from build123d import *

# Parameters (mm, degrees)
BASE_BODY_EXTRUDE_DEPTH         = 25
FLANGE_END_ROUNDS_R12_5_R       = 12.5
EDGE_FILLETS_R6_R               = 6
FLANGE_BOLT_HOLES_2X_DEPTH      = 64.442887702
FLANGE_BOLT_HOLES_2X_DEPTH_BACK = 64.442887702
FLANGE_HOLES_SKETCH_R           = 5
FORK_SLOT_REACH                 = 112.567
FORK_SLOT_DIRECTION_2_DEPTH     = 111.566721937


with BuildPart() as part:
    # Base Profile Sketch → Base Body Extrude (new, symmetric)
    with BuildSketch(Plane.XY):
        with BuildLine():
            Line((50, 40), (50, 0))
            Line((50, 0), (20, 0))
            ThreePointArc((20, 0), (0, 20), (-20, 0))
            Line((-20, 0), (-50, 0))
            Line((-50, 0), (-50, 10))
            Line((-50, 10), (-28.284271247, 10))
            ThreePointArc((-28.284271247, 10), (0, 30), (28.284271247, 10))
            Line((28.284271247, 10), (40, 10))
            Line((40, 10), (40, 40))
            Line((40, 40), (50, 40))
        make_face()
    extrude(amount=BASE_BODY_EXTRUDE_DEPTH, both=True)

    # Flange End Rounds R12.5
    flange_end_rounds_r12_5_edges = [part.edges().sort_by_distance(p)[0] for p in [
        (-50, 5, 25),
        (-50, 5, -25),
    ]]
    fillet(flange_end_rounds_r12_5_edges, radius=FLANGE_END_ROUNDS_R12_5_R)

    # Edge Fillets R6
    edge_fillets_r6_edges = [part.edges().sort_by_distance(p)[0] for p in [
        (45, 40, -25),
        (45, 40, 25),
    ]]
    fillet(edge_fillets_r6_edges, radius=EDGE_FILLETS_R6_R)

    # Flange Holes Sketch → Flange Bolt Holes 2x (cut, two sides: drawn at the far end of the back side and taken through both)
    with BuildSketch(Plane(origin=(0, 10, 0), x_dir=(1, 0, 0), z_dir=(0, 1, 0)).offset(-FLANGE_BOLT_HOLES_2X_DEPTH_BACK)):
        with Locations(Location((-37.5, -12.5, 0), (0, 0, 180))):
            Circle(FLANGE_HOLES_SKETCH_R)
        with Locations(Location((-37.5, 12.5, 0), (0, 0, 180))):
            Circle(FLANGE_HOLES_SKETCH_R)
    extrude(amount=FLANGE_BOLT_HOLES_2X_DEPTH + FLANGE_BOLT_HOLES_2X_DEPTH_BACK, mode=Mode.SUBTRACT)

    # Fork Slot Sketch → Fork Slot (cut, up to next)
    with BuildSketch(Plane(origin=(50, 0, 0), x_dir=(0, 0, -1), z_dir=(1, 0, 0)), mode=Mode.PRIVATE) as fork_slot_sk1:
        with BuildLine():
            Line((7.5, 40), (7.5, 25))
            ThreePointArc((7.5, 25), (0, 17.5), (-7.5, 25))
            Line((-7.5, 25), (-7.5, 40))
            Line((-7.5, 40), (7.5, 40))
        make_face()
    fork_slot_tool1 = extrude(fork_slot_sk1.sketch, amount=-FORK_SLOT_REACH, mode=Mode.PRIVATE) & part.part
    add(fork_slot_tool1.solids().sort_by_distance((50, 29.487689, 0))[0], mode=Mode.SUBTRACT)

    # Fork Slot Sketch → Fork Slot direction 2 (cut)
    with BuildSketch(Plane(origin=(50, 0, 0), x_dir=(0, 0, -1), z_dir=(1, 0, 0))):
        with BuildLine():
            Line((7.5, 40), (7.5, 25))
            ThreePointArc((7.5, 25), (0, 17.5), (-7.5, 25))
            Line((-7.5, 25), (-7.5, 40))
            Line((-7.5, 40), (7.5, 40))
        make_face()
    extrude(amount=FORK_SLOT_DIRECTION_2_DEPTH, mode=Mode.SUBTRACT)


solid = part.part
Read the model definition and answer for the solid it produces. Units are mm, in the model's axes. A direction names the side the tool comes from. Give positions to 0.01 mm unless a question says otherwise; leave off trailing zeros. Write each loop counter-clockwise with the first axis right and the second up, starting at its lowest first coordinate (ties: lowest second). Pieces come first, ordered by that corner, then holes. Notation, with made-up numbers: (75.5, 11) - (91.5, 11) arc R19 ccw to (91.5, 20) - close; hole circle Ø1 at (67, 19.25). An arc over 180 degrees is marked (long way). Answer in a Markdown table with one row per item. Add a question column.
Item 1: Determine the mould class of faces 1 (the face through (45.07, 38.196, 23.289)), 2 (the face through (0, 20, 0)), 3 (the face through (-32.505, 4.93, 12.72)) for opening direction Z: pulls with the +Z half, pulls with the -Z half, needs draft (parallel to the pull), parting line crosses it, or undercut.
Item 2: Section A-A, the plane z = 8.5 is taken. Write down the section's boundary in (x, y), and give its area (3 significant figures).
Item 3: Section B-B, the plane y = 31 is taken. Write down the section's boundary in (x, z), and give its area (3 significant figures).
Item 4: A tool of negligible diameter and unlimited length cuts with its end or side. For faces 4 (the face through (45.07, 38.289, -23.196)), 5 (the face through (45, 33, -7.5)), 6 (the face through (40, 18, 6)), from which of +Z, -Z, +X, -X, +Y, -Y can it reach the whole face along a straight path? Write none if from no direction.
Item 5: Section C-C, the plane x = -36 is taken. Write down the section's boundary in (y, z), and give its area (3 significant figures).
Item 6: Section D-D, the plane y = 22.5 is taken. Write down the section's boundary in (x, z).
Item 7: Find the intervals of material crossed by L1, parallel to Z at x = -37.5, y = 6.5; L2, parallel to X at y = 3.75, z = -12.5; L3, parallel to X at y = 6, z = 16, in increasing order.
Item 8: Flat-ended cylindrical pins translate along their axes: P1, Ø8, axis at x = -10, y = 32, coming from the -Z side; P2, Ø1, axis at y = 36, z = -8, coming from the -X side; P3, Ø13, axis at x = 32.5, z = 5, coming from the +Y side; P4, Ø11, axis at x = -36, z = 4, coming from the +Y side. Find the tip coordinate at first contact, or state that the pin passes through.
Recorded:
| question | item | result |
|---|---|---|
| 1 | face 1 | pulls with the +Z half |
| 1 | face 2 | needs draft |
| 1 | face 3 | undercut |
| 2 | outline | (-50, 0) - (-40.5, 0) - (-40.5, 10) - (-50, 10) - close; (-34.5, 0) - (-20, 0) arc R20 cw to (20, 0) - (50, 0) - (50, 40) - (40, 40) - (40, 10) - (28.28, 10) arc R30 ccw to (-28.28, 10) - (-34.5, 10) - close |
| 2 | area | 1,440 mm2 |
| 3 | outline | (40, -25) - (50, -25) - (50, -7.5) - (40, -7.5) - close; (40, 7.5) - (50, 7.5) - (50, 25) - (40, 25) - close |
| 3 | area | 350 mm2 |
| 4 | face 4 | -Z, +X, -X, +Y |
| 4 | face 5 | +X, +Y |
| 4 | face 6 | +Z, -Z, +Y |
| 5 | outline | (0, -25) - (10, -25) - (10, -17.27) - (0, -17.27) - close; (0, -7.73) - (10, -7.73) - (10, 7.73) - (0, 7.73) - close; (0, 17.27) - (10, 17.27) - (10, 25) - (0, 25) - close |
| 5 | area | 309 mm2 |
| 6 | outline | (-19.84, -25) - (19.84, -25) - (19.84, 25) - (-19.84, 25) - close; (40, -25) - (50, -25) - (50, -7.07) - (40, -7.07) - close; (40, 7.07) - (50, 7.07) - (50, 25) - (40, 25) - close |
| 7 | L1 | z = -25 to -17.5, -7.5 to 7.5, 17.5 to 25 |
| 7 | L2 | x = -50 to -42.5, -32.5 to -19.65, 19.65 to 50 |
| 7 | L3 | x = -49.5 to -41.07, -33.93 to -19.08, 19.08 to 50 |
| 8 | P1 | stops at z = -25 |
| 8 | P2 | stops at x = 40 |
| 8 | P3 | stops at y = 14.97 |
| 8 | P4 | stops at y = 10 |
